Input: part model. Units: mm. Frame: model coordinates. Face numbers are marked on the shaded views. A direction names the side the tool comes from. Coordinates: 2 decimals unless noted, no trailing zeros. Loops run counter-clockwise (first coordinate to the right, second up) from the corner with the lowest first, then second, coordinate; pieces in that order, holes last. Notation, with made-up numbers: (40.5, 53.5) -> (55.5, 53.5) arc R4 ccw to (55.5, 60.5) -> close; hole circle Ø5 at (-25.5, 11). An arc over 180 degrees is marked (long way). Answer as a JSON object with one key per item and string values.
from build123d import *

# Parameters (mm, degrees)
SKETCH_1_W          = 90
SKETCH_1_H          = 50
EXTRUDE_1_DEPTH     = 4
SKETCH_2_R          = 5.5
CUT_EXTRUDE_1_DEPTH = 52.633322574
SKETCH_3_W          = 100
SKETCH_3_H          = 80
SKETCH_3_R          = 5.5
EXTRUDE_2_DEPTH     = 10
SKETCH_4_R          = 5.5
CUT_EXTRUDE_2_DEPTH = 82.492330928


with BuildPart() as part:
    # 草图1 → 凸台-拉伸1 (new body)
    with BuildSketch(Plane.XY):
        Rectangle(SKETCH_1_W, SKETCH_1_H)
    extrude_1 = extrude(amount=EXTRUDE_1_DEPTH)

    # 草图2 → 切除-拉伸1 (cut, through all)
    with BuildSketch(Plane.XY.offset(4)):
        with Locations((-10, 0)):
            Circle(SKETCH_2_R)
        with Locations((10, 0)):
            Circle(SKETCH_2_R)
    extrude(amount=-CUT_EXTRUDE_1_DEPTH, mode=Mode.SUBTRACT)

    # 草图3 → 凸台-拉伸2 (add)
    with BuildSketch(Plane.XZ.offset(25)):
        with Locations((0, -14)):
            Rectangle(SKETCH_3_W, SKETCH_3_H)
        with Locations(Location((-35, 16, 0), (0, 0, 270))):
            Circle(SKETCH_3_R, mode=Mode.SUBTRACT)
        with Locations(Location((35, 16, 0), (0, 0, 270))):
            Circle(SKETCH_3_R, mode=Mode.SUBTRACT)
        with Locations(Location((35, -44, 0), (0, 0, 270))):
            Circle(SKETCH_3_R, mode=Mode.SUBTRACT)
        with Locations(Location((-35, -44, 0), (0, 0, 270))):
            Circle(SKETCH_3_R, mode=Mode.SUBTRACT)
    extrude(amount=EXTRUDE_2_DEPTH)

    # 镜向1: 凸台-拉伸1 across plane
    add(extrude_1.mirror(Plane(origin=(0, 0, -14), x_dir=(1, 0, 0), z_dir=(0, 0, -1))))

    # 草图4 → 切除-拉伸2 (cut, through all)
    with BuildSketch(Plane.XY.offset(-28)):
        with Locations((-10, 0)):
            Circle(SKETCH_4_R)
        with Locations((10, 0)):
            Circle(SKETCH_4_R)
    extrude(amount=-CUT_EXTRUDE_2_DEPTH, mode=Mode.SUBTRACT)


solid = part.part
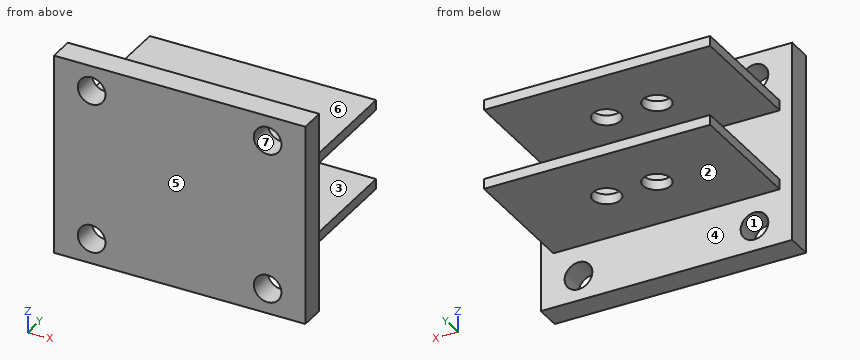
1. Section query C-C (y = 15.5). Return loops of the section in (x, z).
Reply:
{"outline": "(-45, -32) -> (45, -32) -> (45, -28) -> (-45, -28) -> close; (-45, 0) -> (45, 0) -> (45, 4) -> (-45, 4) -> close"}
2. Section query A-A (z = -44). Return loops of the section in (x, y).
Reply:
{"outline": "(-50, -35) -> (-40.5, -35) -> (-40.5, -25) -> (-50, -25) -> close; (-29.5, -35) -> (29.5, -35) -> (29.5, -25) -> (-29.5, -25) -> close; (40.5, -35) -> (50, -35) -> (50, -25) -> (40.5, -25) -> close"}
3. Section query D-D (y = 0). Return loops of the section in (x, z).
Reply:
{"outline": "(-45, -32) -> (-15.5, -32) -> (-15.5, -28) -> (-45, -28) -> close; (-45, 0) -> (-15.5, 0) -> (-15.5, 4) -> (-45, 4) -> close; (-4.5, -32) -> (4.5, -32) -> (4.5, -28) -> (-4.5, -28) -> close; (-4.5, 0) -> (4.5, 0) -> (4.5, 4) -> (-4.5, 4) -> close; (15.5, -32) -> (45, -32) -> (45, -28) -> (15.5, -28) -> close; (15.5, 0) -> (45, 0) -> (45, 4) -> (15.5, 4) -> close"}
4. Mould query, pull axis Z, two halves, no side actions, for the marked faces 4, 5, 6 and 7. Classes: pulls with the +Z half, pulls with the -Z half, needs draft (parallel to the pull), parting line crosses it, or undercut.
Reply:
{"face 4": "undercut", "face 5": "needs draft", "face 6": "pulls with the +Z half", "face 7": "undercut"}
5. Access query for the marked faces 1, 2 and 3. Directions: +Z, -Z, +X, -X, +Y, -Y. A direction counts if a zero-diameter tool reaches every point of the face in a straight line with its end or side. Return the directions, or none.
Reply:
{"face 1": "+Y, -Y", "face 2": "-Z, +X, -X, +Y", "face 3": "+X, -X, +Y"}
6. Line query: line 1 along Z through (x, y) = (12, 10); line 2 along Z through (x, y) = (-34, -32.5); line 3 along Y through (x, z) = (10, -28.85). Output: solid intervals per line, ascending.
Reply:
{"line 1": "z = -32 to -28, 0 to 4", "line 2": "z = -54 to -49.41, -38.59 to 10.59, 21.41 to 26", "line 3": "y = -35 to -5.5, 5.5 to 25"}
7. Section query B-B (x = 10). Return loops of the section in (y, z).
Reply:
{"outline": "(-35, -54) -> (-25, -54) -> (-25, -32) -> (-5.5, -32) -> (-5.5, -28) -> (-25, -28) -> (-25, 0) -> (-5.5, 0) -> (-5.5, 4) -> (-25, 4) -> (-25, 26) -> (-35, 26) -> close; (5.5, -32) -> (25, -32) -> (25, -28) -> (5.5, -28) -> close; (5.5, 0) -> (25, 0) -> (25, 4) -> (5.5, 4) -> close"}
8. Pin query (flat end, axial travel): P1, Ø8, axis at y = 5, z = -2, coming from the -X side; P2, Ø9, axis at x = -35, z = 16, coming from the +Y side; P3, Ø15, axis at x = -9.5, y = -12.5, coming from the -Z side; P4, Ø17.5, axis at x = 35, z = 16, coming from the +Y side. Return the tip coordinate at first contact, or that it passes through.
Reply:
{"P1": "stops at x = -45", "P2": "passes through", "P3": "stops at z = -32", "P4": "stops at y = -25"}
